Source: CAD feature listing. Evaluate the final solid. Frame: model axes, mm. Give positions to 0.01 mm unless a question says otherwise; leave off trailing zeros. Order: outer loops, then holes, each group sorted by start corner. A loop starts at its lowest first (then second) coordinate and runs counter-clockwise, first axis right, second up. Notation, with made-up numbers: (87, -39.75) - (95, -39.75) arc R12 ccw to (95, -33.75) - close; hole circle Ø11 at (2, 45). An arc over 180 degrees is marked (long way). Write each question's results on one line, items separated by ' | '. Start each with the question number.
Item 1: Line query: line 1 along X through (y, z) = (20.5, -22.5); line 2 along X through (y, z) = (6, 12). Output: solid intervals per line, ascending.
Item 2: Section B-B on y = 22.25. Output: boundary loops of the cut face in (x, z), and give its area (3 significant figures).
Item 3: Contact query for flat-ended pins moving along their axis: pin 1 Ø11 at (y, z) = (16, -108) entering from +X; pin 2 Ø17 at (x, z) = (20, 8.5) entering from +Y. Output: stop coordinate, or through.
Item 4: Section A-A on z = 15. Output: boundary loops of the cut face in (x, y), and give its area (3 significant figures).
```python
from build123d import *

# Parameters (mm, degrees)
BOSS_EXTRUDE1_DEPTH = 219.4


with BuildPart() as part:
    # Sketch1 → Boss-Extrude1 (new, symmetric)
    with BuildSketch(Plane.XY):
        with BuildLine():
            Line((0, 0), (0, 30))
            Line((0, 30), (2, 30))
            ThreePointArc((2, 30), (2.707106781, 29.707106781), (3, 29))
            Line((3, 29), (3, 7.5))
            ThreePointArc((3, 7.5), (4.318019485, 4.318019485), (7.5, 3))
            Line((7.5, 3), (29, 3))
            ThreePointArc((29, 3), (29.707106781, 2.707106781), (30, 2))
            Line((30, 2), (30, 0))
            Line((30, 0), (0, 0))
        make_face()
    extrude(amount=BOSS_EXTRUDE1_DEPTH, both=True)


solid = part.part
```
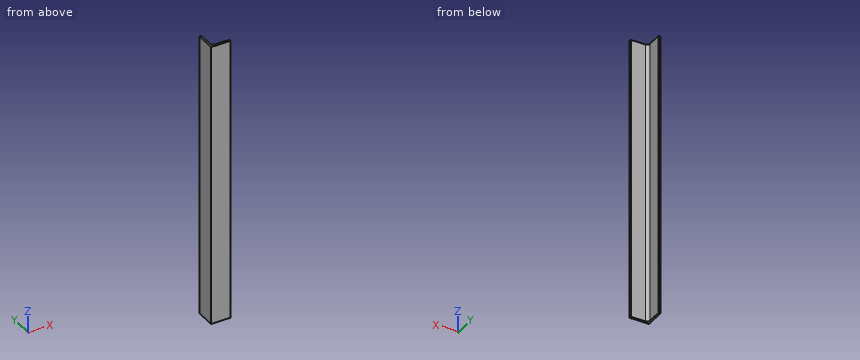
Evaluation:
1) line 1: x = 0 to 3 | line 2: x = 0 to 3.26
2) outline: (0, -219.4) - (3, -219.4) - (3, 219.4) - (0, 219.4) - close | area: 1,320 mm^2
3) pin 1: stops at x = 3 | pin 2: stops at y = 3
4) outline: (0, 0) - (30, 0) - (30, 2) arc R1 ccw to (29, 3) - (7.5, 3) arc R4.5 cw to (3, 7.5) - (3, 29) arc R1 ccw to (2, 30) - (0, 30) - close | area: 175 mm^2
